Build history of the part. All positions in model axes, mm. Give positions to 0.01 mm unless a question says otherwise; leave off trailing zeros. Order: outer loops, then holes, each group sorted by start corner. A loop starts at its lowest first (then second) coordinate and runs counter-clockwise, first axis right, second up. Notation, with made-up numbers: (26.5, 68.25) - (80.5, 68.25) arc R21 ccw to (80.5, 107.25) - close; hole circle Ø7 at (84.5, 16). An arc over 180 degrees is marked (long way). Write each question's results on one line, items separated by ' | '. Start each with the question number.
1) Cut at A-A on x = 200. List the corners of the cut face in (y, z).
2) Drop flat-ended pins along their axis: pin 1 Ø4.5 at (x, y) = (225.5, 2.5) entering from -Z; pin 2 Ø5.5 at (x, z) = (-278.5, 77) entering from +Y. Give the stop position or say it passes through.
3) Drill centre lines: line 1 along X through (y, z) = (4, 20); line 2 along X through (y, z) = (-4, -15); line 3 along X through (y, z) = (-3.75, 75). Where is each one in solid material? Low to high. Write a range as from..to.
from build123d import *

# Parameters (mm, degrees)
SKETCH_1_W                   = 570
SKETCH_1_H                   = 350
EXTRUDE_1_DEPTH              = 7.5
CHAMFER_1_SIZE               = 5
HOLE_WIZARD_M5_1_D           = 4.2
HOLE_WIZARD_M8_1_D           = 6.8
HOLE_WIZARD_M6_1_D           = 6.6
HOLE_WIZARD_M6_1_DEPTH       = 17
HOLE_WIZARD_M6_1_CBORE_D     = 11
HOLE_WIZARD_M6_1_CBORE_DEPTH = 6.4
HOLE_WIZARD_M6_1_TIP         = 1.982840043
HOLE_WIZARD_M6_2_D           = 6.6
HOLE_WIZARD_M6_2_DEPTH       = 17
HOLE_WIZARD_M6_2_CBORE_D     = 11
HOLE_WIZARD_M6_2_CBORE_DEPTH = 6.4
HOLE_WIZARD_M6_2_TIP         = 1.982840043
SKETCH_10_W                  = 120
SKETCH_10_H                  = 120
CUT_EXTRUDE_1_DEPTH          = 335.776044543
FILLET_1_R                   = 10
CHAMFER_2_SIZE               = 5


with BuildPart() as part:
    # 草图1 → 凸台-拉伸1 (new, symmetric)
    with BuildSketch(Plane(origin=(0, 0, 0), x_dir=(1, 0, 0), z_dir=(0, 1, 0))):
        Rectangle(SKETCH_1_W, SKETCH_1_H)
    extrude(amount=EXTRUDE_1_DEPTH, both=True)

    # 倒角1
    chamfer_1_edges = [part.edges().sort_by_distance(p)[0] for p in [
        (-285, 0, -175),
        (285, 0, -175),
        (285, 0, 175),
        (-285, 0, 175),
    ]]
    chamfer(chamfer_1_edges, length=CHAMFER_1_SIZE)

    # M5 螺纹孔1 (through all)
    with Locations(Plane(origin=(0, 7.5, 0), x_dir=(1, 0, 0), z_dir=(0, 1, 0))):
        with Locations((-265, 125), (-235, 95), (-235, 155), (-205, 125)):
            Hole(HOLE_WIZARD_M5_1_D / 2)

    # M8 螺纹孔1 (through all)
    with Locations(Plane(origin=(0, 7.5, 0), x_dir=(1, 0, 0), z_dir=(0, 1, 0))):
        with Locations((85, -20), (127, -20), (127, 160), (85, 160)):
            Hole(HOLE_WIZARD_M8_1_D / 2)

    # M6 六角凹头螺钉的柱形沉头孔1
    with Locations(Plane(origin=(0, 7.5, 0), x_dir=(1, 0, 0), z_dir=(0, 1, 0))):
        with Locations((-277.5, 15), (-277.5, -165), (277.5, 15), (277.5, -165), (-277.5, -75), (277.5, -75)):
            CounterBoreHole(HOLE_WIZARD_M6_1_D / 2, HOLE_WIZARD_M6_1_CBORE_D / 2, HOLE_WIZARD_M6_1_CBORE_DEPTH, depth=HOLE_WIZARD_M6_1_DEPTH)
            with Locations((0, 0, -(HOLE_WIZARD_M6_1_DEPTH + HOLE_WIZARD_M6_1_TIP / 2))):  # 118° drill point
                Cone(0, HOLE_WIZARD_M6_1_D / 2, HOLE_WIZARD_M6_1_TIP, mode=Mode.SUBTRACT)

    # M6 六角凹头螺钉的柱形沉头孔2
    with Locations(Plane(origin=(0, 7.5, 0), x_dir=(1, 0, 0), z_dir=(0, 1, 0))):
        with Locations((-245, -75), (245, -75)):
            CounterBoreHole(HOLE_WIZARD_M6_2_D / 2, HOLE_WIZARD_M6_2_CBORE_D / 2, HOLE_WIZARD_M6_2_CBORE_DEPTH, depth=HOLE_WIZARD_M6_2_DEPTH)
            with Locations((0, 0, -(HOLE_WIZARD_M6_2_DEPTH + HOLE_WIZARD_M6_2_TIP / 2))):  # 118° drill point
                Cone(0, HOLE_WIZARD_M6_2_D / 2, HOLE_WIZARD_M6_2_TIP, mode=Mode.SUBTRACT)

    # 草图10 → 切除-拉伸1 (cut, through all)
    with BuildSketch(Plane(origin=(0, 7.5, 0), x_dir=(1, 0, 0), z_dir=(0, 1, 0))):
        with Locations((225, 115)):
            Rectangle(SKETCH_10_W, SKETCH_10_H)
    extrude(amount=-CUT_EXTRUDE_1_DEPTH, mode=Mode.SUBTRACT)

    # 圆角1
    fillet_1_edges = [part.edges().sort_by_distance(p)[0] for p in [
        (165, 0, -55),
    ]]
    fillet(fillet_1_edges, radius=FILLET_1_R)

    # 倒角2
    chamfer_2_edges = [part.edges().sort_by_distance(p)[0] for p in [
        (285, 0, -55),
        (165, 0, -175),
    ]]
    chamfer(chamfer_2_edges, length=CHAMFER_2_SIZE)


solid = part.part
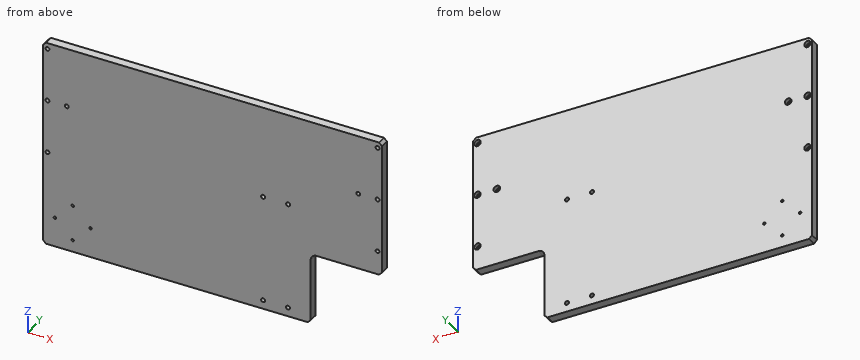
Results:
1) outline: (-7.5, -55) - (7.5, -55) - (7.5, 175) - (-7.5, 175) - close
2) pin 1: z = -55 | pin 2: y = 1.1
3) line 1: -285..81.6, 88.4..123.6, 130.4..285 | line 2: -285..-280.8, -274.2..274.2, 280.8..285 | line 3: -285..-280.8, -274.2..-248.3, -241.7..241.7, 248.3..274.2, 280.8..285
